The figure shows three views and two pictorial views of one solid part (mm, origin at its lowest corner). Answer the questions. A direction names the side the tool comes from. Coordinates: 2 decimals unless noted, no trailing zeros. Order: outer loops, then holes, each group sorted by start corner. A loop starts at its lowest first (then second) coordinate and runs counter-clockwise, first axis right, second up. Notation, with made-up numbers: (60.5, -20.75) - (77.5, -20.75) arc R11 cw to (77.5, -14.75) - close; hole circle Ø2 at (57.25, -3.75). An arc over 180 degrees is marked (long way). Answer as a JSON object with one key per item and string values. Group by question number.
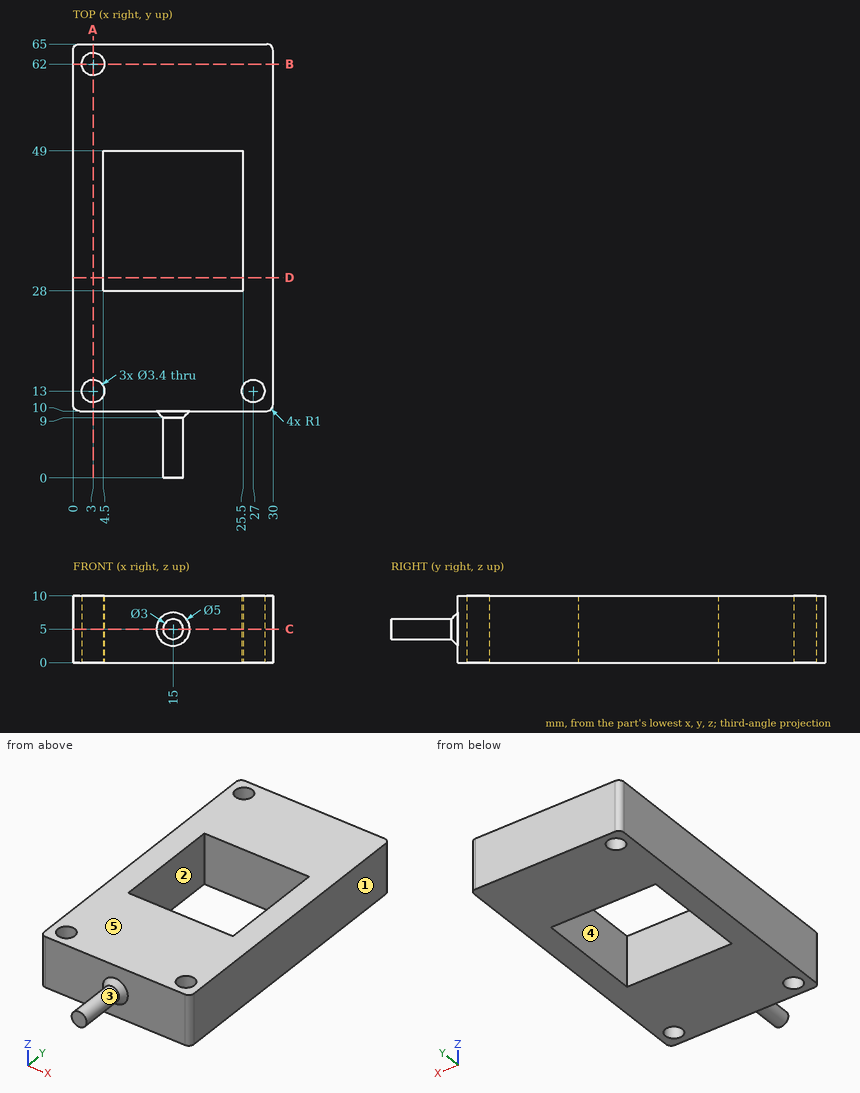
1. A cutting plane is placed at D-D on y = 30. Write down the section's boundary in (x, z).
2. A cutting plane is placed at C-C on z = 5. Write down the section's boundary in (x, y), and give its area (3 significant figures).
3. A cutting plane is placed at B-B on y = 62. Write down the section's boundary in (x, z).
4. Straight lines are drawn through the part: L1, parallel to Y at x = 3, z = 3.75; L2, parallel to Y at x = 9, z = 8.25; L3, parallel to X at y = 48, z = 2.75. For each, find the intervals that lie inside material, in ascending order.
5. For the marked faces 1 and 2, determine the directions among +Z, -Z, +X, -X, +Y, -Y from which every point of the face is accessible in a straight line to the end or side of a thin tool.
6. For a pull along X with two mould halves and no side action, classify the marked faces 3, 4 and 5 as pulls with the +X half, pulls with the -X half, needs draft (parallel to the pull), parting line crosses it, or undercut.
7. A cutting plane is placed at A-A on x = 3. Write down the section's boundary in (y, z), and give its area (3 significant figures).
8. Given pin 1 (2.5 mm diameter, centred on x = 3, y = 62, fed in from -Z); pin 2 (3 mm diameter, centred on x = 11, z = 6, fed in from -Y), each flat-ended and moving along its own axis, determine where each tip first touches the part or whether it passes through.
Derived:
{
 "1": {"outline": "(0, 0) - (4.5, 0) - (4.5, 10) - (0, 10) - close; (25.5, 0) - (30, 0) - (30, 10) - (25.5, 10) - close"},
 "2": {"outline": "(0, 11) arc R1 ccw to (1, 10) - (12.5, 10) - (13.5, 9) - (13.5, 0) - (16.5, 0) - (16.5, 9) - (17.5, 10) - (29, 10) arc R1 ccw to (30, 11) - (30, 64) arc R1 ccw to (29, 65) - (1, 65) arc R1 ccw to (0, 64) - close; hole circle Ø3.4 at (3, 13); hole circle Ø3.4 at (3, 62); hole (4.5, 28) - (25.5, 28) - (25.5, 49) - (4.5, 49) - close; hole circle Ø3.4 at (27, 13)", "area": "1,210 mm2"},
 "3": {"outline": "(0, 0) - (1.3, 0) - (1.3, 10) - (0, 10) - close; (4.7, 0) - (30, 0) - (30, 10) - (4.7, 10) - close"},
 "4": {"L1": "y = 10 to 11.3, 14.7 to 60.3, 63.7 to 65", "L2": "y = 10 to 28, 49 to 65", "L3": "x = 0 to 4.5, 25.5 to 30"},
 "5": {"face 1": "+Z, -Z, +X, +Y, -Y", "face 2": "+Z, -Z"},
 "6": {"face 3": "parting line crosses it", "face 4": "undercut", "face 5": "needs draft"},
 "7": {"outline": "(10, 0) - (11.3, 0) - (11.3, 10) - (10, 10) - close; (14.7, 0) - (60.3, 0) - (60.3, 10) - (14.7, 10) - close; (63.7, 0) - (65, 0) - (65, 10) - (63.7, 10) - close", "area": "482 mm2"},
 "8": {"pin 1": "passes through", "pin 2": "stops at y = 10"}
}
